from build123d import *

# Parameters (mm, degrees)
BLADE_FLAT_CUT_DEPTH = 10


with BuildPart() as part:
    # Shaft Profile Sketch → Shaft Revolve (revolve)
    with BuildSketch(Plane.XY, mode=Mode.PRIVATE) as shaft_revolve_sk:
        Polygon((0, 0), (0, 3), (76, 3), (96, 6), (108, 3.5), (108, 0), align=None)
    revolve(shaft_revolve_sk.sketch.rotate(Axis((-206.404998063, 0, 0), (1, 0, 0)), 90), axis=Axis((-206.404998063, 0, 0), (1, 0, 0)))

    # Blade Flat Sketch → Blade Flat Cut (cut, symmetric)
    with BuildSketch(Plane(origin=(0, 0, 0), x_dir=(1, 0, 0), z_dir=(0, 1, 0))):
        Polygon((108, 1), (76, 3), (76, 10.728035522), (108, 10.728035522), align=None)
    blade_flat_cut = extrude(amount=BLADE_FLAT_CUT_DEPTH, both=True, mode=Mode.SUBTRACT)

    # Blade Flat Mirror: Blade Flat Cut across plane
    add(blade_flat_cut.mirror(Plane.XY), mode=Mode.SUBTRACT)


solid = part.part
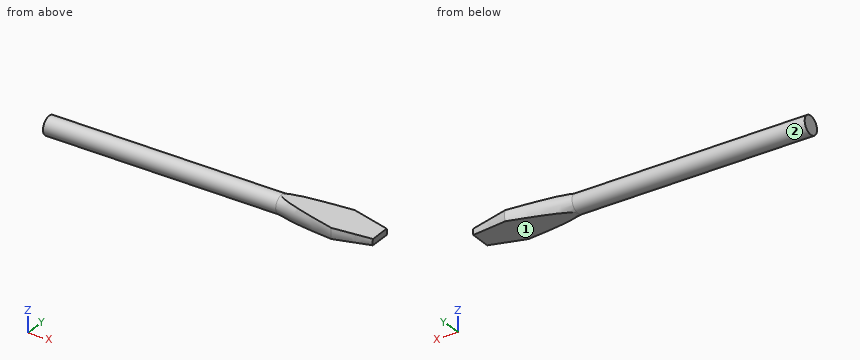
Design review of the part built by this model. Coordinates are the model's own, in mm. Face numbers are marked on the shaded views. A direction names the side the tool comes from. Give positions to 0.01 mm unless a question says otherwise; leave off trailing zeros. Order: outer loops, then holes, each group sorted by start corner. A loop starts at its lowest first (then second) coordinate and runs counter-clockwise, first axis right, second up.
1. For pin 1 Ø1.5 at (x, z) = (97, 0.5) entering from +Y; pin 2 Ø2 at (y, z) = (3, 2) entering from -X, all flat-tipped, find the tip position at first contact; note any pin that passes through.
Solution:
pin 1: stops at y = 5.93
pin 2: stops at x = 0
2. Add section B-B, the plane x = 14. State the section outline as (y, z) points, then the cut area to 3 significant figures.
Solution:
outline: circle Ø6 at (0, 0)
area: 28.3 mm2
3. Add section A-A, the plane z = 0. State the section outline as (x, y) points, then the cut area to 3 significant figures.
Solution:
outline: (0, -3) - (76, -3) - (96, -6) - (108, -3.5) - (108, 3.5) - (96, 6) - (76, 3) - (0, 3) - close
area: 750 mm2
4. Tool access review of the marked faces 1 and 2: name each direction out of +Z, -Z, +X, -X, +Y, -Y from which nothing blocks a thin tool from reaching the whole face with its end or side.
Solution:
face 1: -Z, +X, +Y, -Y
face 2: -X
5. To check wall thickness, follow L1, parallel to Y at x = 70, z = 0.15; L2, parallel to Y at x = 44, z = -1; L3, parallel to Z at x = 65, y = 2.75. State the ranges of each line that lie inside material, in increasing order.
Solution:
L1: y = -3 to 3
L2: y = -2.83 to 2.83
L3: z = -1.2 to 1.2
6. Add section C-C, the plane x = 101. State the section outline as (y, z) points, then the cut area to 3 significant figures.
Solution:
outline: (-4.75, -1.44) - (4.75, -1.44) arc R4.96 ccw to (4.75, 1.44) - (-4.75, 1.44) arc R4.96 ccw to start
area: 28.1 mm2
